Geometry check sheet. Reference: the model listing, model coordinates, mm. A direction names the side the tool comes from. Give positions to 0.01 mm unless a question says otherwise; leave off trailing zeros. Write each loop counter-clockwise with the first axis right and the second up, starting at its lowest first coordinate (ties: lowest second). Pieces come first, ordered by that corner, then holes. Notation, with made-up numbers: (-4, -33) -> (48, -33) arc R23 ccw to (48, -15) -> close; hole circle Ø5 at (-28.5, 69). An arc over 180 degrees is marked (long way). One line per item, written item: value.
from build123d import *

# Parameters (mm, degrees)
SKETCH_1_R          = 125
SKETCH_1_R_2        = 5.25
EXTRUDE_1_DEPTH     = 42.13
SKETCH_2_R          = 65
EXTRUDE_2_DEPTH     = 15
SKETCH_3_R          = 30
CUT_EXTRUDE_1_DEPTH = 55
SKETCH_6_R          = 5
CUT_EXTRUDE_2_DEPTH = 50
SKETCH_7_R          = 9
CUT_EXTRUDE_3_DEPTH = 11


with BuildPart() as part:
    # 草图1 → 凸台-拉伸1 (new body)
    with BuildSketch(Plane.XY):
        Circle(SKETCH_1_R)
        with Locations((0, 90)):
            Circle(SKETCH_1_R_2, mode=Mode.SUBTRACT)
        with Locations((63.639610307, 63.639610307)):
            Circle(SKETCH_1_R_2, mode=Mode.SUBTRACT)
        with Locations((90, 0)):
            Circle(SKETCH_1_R_2, mode=Mode.SUBTRACT)
        with Locations((63.639610307, -63.639610307)):
            Circle(SKETCH_1_R_2, mode=Mode.SUBTRACT)
        with Locations((0, -90)):
            Circle(SKETCH_1_R_2, mode=Mode.SUBTRACT)
        with Locations((-63.639610307, -63.639610307)):
            Circle(SKETCH_1_R_2, mode=Mode.SUBTRACT)
        with Locations((-90, 0)):
            Circle(SKETCH_1_R_2, mode=Mode.SUBTRACT)
        with Locations((-63.639610307, 63.639610307)):
            Circle(SKETCH_1_R_2, mode=Mode.SUBTRACT)
    extrude(amount=EXTRUDE_1_DEPTH)

    # 草图2 → 凸台-拉伸2 (add)
    with BuildSketch(Plane.XY.offset(42.13)):
        Circle(SKETCH_2_R)
    extrude(amount=EXTRUDE_2_DEPTH)

    # 草图3 → 切除-拉伸1 (cut)
    with BuildSketch(Plane.XY.offset(57.13)):
        Circle(SKETCH_3_R)
    extrude(amount=-CUT_EXTRUDE_1_DEPTH, mode=Mode.SUBTRACT)

    # 草图5 → 切除-旋转1 (revolve, cut)
    with BuildSketch(Plane(origin=(0, 0, 0), x_dir=(0, 0, 1), z_dir=(-0.3826834323650906, 0.9238795325112865, 0)), mode=Mode.PRIVATE) as cut_revolve_1_sk:
        Polygon((30, 100.5), (37.70842723, 127.382480462), (25, 127.382480462), (25, 124.917518293), (25, 0), (30, 0), align=None)
    revolve(cut_revolve_1_sk.sketch.rotate(Axis((123.47749494, 51.146053052, 25), (-0.9238795325112864, -0.3826834323650906, 0)), 90), axis=Axis((123.47749494, 51.146053052, 25), (-0.9238795325112864, -0.3826834323650906, 0)), mode=Mode.SUBTRACT)

    # 草图6 → 切除-拉伸2 (cut)
    with BuildSketch(Plane.XY.offset(42.13)):
        with Locations((43.884277794, 18.177463037)):
            Circle(SKETCH_6_R)
    extrude(amount=-CUT_EXTRUDE_2_DEPTH, mode=Mode.SUBTRACT)

    # 草图7 → 切除-拉伸3 (cut)
    with BuildSketch(Plane(origin=(0, 0, 0), x_dir=(-1, 0, 0), z_dir=(0, 0, -1))):
        with Locations((0, 90)):
            Circle(SKETCH_7_R)
        with Locations((63.639610307, 63.639610307)):
            Circle(SKETCH_7_R)
        with Locations((90, 0)):
            Circle(SKETCH_7_R)
        with Locations((63.639610307, -63.639610307)):
            Circle(SKETCH_7_R)
        with Locations((0, -90)):
            Circle(SKETCH_7_R)
        with Locations((-63.639610307, -63.639610307)):
            Circle(SKETCH_7_R)
        with Locations((-90, 0)):
            Circle(SKETCH_7_R)
        with Locations((-63.639610307, 63.639610307)):
            Circle(SKETCH_7_R)
    extrude(amount=-CUT_EXTRUDE_3_DEPTH, mode=Mode.SUBTRACT)


solid = part.part
1) Sectioned sample at A-A on x = 0. Record the cut outline in (y, z).
Verdict:
outline: (-125, 0) -> (-99, 0) -> (-99, 11) -> (-95.25, 11) -> (-95.25, 42.13) -> (-125, 42.13) -> close; (-84.75, 11) -> (-81, 11) -> (-81, 0) -> (81, 0) -> (81, 11) -> (84.75, 11) -> (84.75, 42.13) -> (65, 42.13) -> (65, 57.13) -> (30, 57.13) -> (30, 2.13) -> (-30, 2.13) -> (-30, 57.13) -> (-65, 57.13) -> (-65, 42.13) -> (-84.75, 42.13) -> close; (95.25, 11) -> (99, 11) -> (99, 0) -> (125, 0) -> (125, 42.13) -> (95.25, 42.13) -> close
2) Sectioned sample at C-C on x = -90. Record the cut outline in (y, z).
Verdict:
outline: (-86.75, 0) -> (-9, 0) -> (-9, 11) -> (-5.25, 11) -> (-5.25, 42.13) -> (-86.75, 42.13) -> close; (5.25, 11) -> (9, 11) -> (9, 0) -> (86.75, 0) -> (86.75, 42.13) -> (5.25, 42.13) -> close
3) Mould release check, pull along Z, two halves, no side actions. Record for faces 4 (the cylindrical face through (81.416, 2.703, 5.423)), 5 (the cylindrical face through (32.058, 18.441, 23.498)), 6 (the flat face through (0, 0, 2.13)): released by +Z, released by -Z, zero draft, split by the parting line, or undercut.
Verdict:
face 4: zero draft
face 5: undercut
face 6: released by +Z
4) Depth check by flat-ended pin: pin 1 Ø13.5 at (x, y) = (63.64, -63.64) entering from -Z; pin 2 Ø2 at (x, y) = (-89, -43.5) entering from +Z; pin 3 Ø2 at (y, z) = (91.5, 9) entering from -X (3 decimals); pin 4 Ø8.5 at (x, y) = (-90, 0) entering from +Z. Enter the tip coordinate at first touch or a pass-through.
Verdict:
pin 1: z = 11
pin 2: z = 42.13
pin 3: x = -86.225
pin 4: through
5) Tool access check on faces 1 (the cylindrical face through (68.647, -62.063, 26.347)), 2 (the flat face through (60, -68, 11)), 3 (the cylindrical face through (-29.97, 1.32, 30.02)). Record the directions out of +Z, -Z, +X, -X, +Y, -Y that give a thin tool (end or side, any length) a straight path to the whole face; none if there is none.
Verdict:
face 1: +Z, -Z
face 2: -Z
face 3: +Z
6) Sectioned sample at B-B on z = 45. Record the cut outline in (x, y), plus the area to 3 significant figures.
Verdict:
outline: circle Ø130 at (0, 0); hole circle Ø60 at (0, 0)
area: 10,400 mm^2
7) Scan lines: probe 1 along Y at (x, z) = (0, 8); probe 2 along Z at (x, y) = (93.5, -36); probe 3 along Y at (x, z) = (56.5, 10). Record each from-to range of solid material in increasing order.
Verdict:
probe 1: -125 to -99, -81 to -30, 30 to 81, 99 to 125
probe 2: 0 to 42.13
probe 3: -111.5 to -69.12, -58.16 to 58.16, 69.12 to 111.5
